from build123d import *

# Parameters (mm, degrees)
SKETCH_1_W      = 38
SKETCH_1_H      = 80
EXTRUDE_1_DEPTH = 4
SKETCH_2_W      = 38
SKETCH_2_H      = 8
EXTRUDE_2_DEPTH = 16


with BuildPart() as part:
    # 草图1 → 凸台-拉伸1 (new, symmetric)
    with BuildSketch(Plane.XY):
        Rectangle(SKETCH_1_W, SKETCH_1_H)
    extrude(amount=EXTRUDE_1_DEPTH, both=True)

    # 草图2 → 凸台-拉伸2 (add)
    with BuildSketch(Plane.XY.offset(4)):
        with Locations((0, 36)):
            Rectangle(SKETCH_2_W, SKETCH_2_H)
    extrude(amount=EXTRUDE_2_DEPTH)


solid = part.part
Work out the finished part from the listing and answer in its coordinate system (mm). A direction names the side the tool comes from. Coordinates: 2 decimals unless noted, no trailing zeros. Loops run counter-clockwise (first coordinate to the right, second up) from the corner with the lowest first, then second, coordinate; pieces in that order, holes last. Notation, with made-up numbers: M 46.5,35.25 L 90.5,35.25 A38 cw 90.5,74.25 Z; hole C -25,54 d9. An arc over 180 degrees is marked long. Answer in a Markdown table with one row per item. Add a question column.
1. A tool of negligible diameter and unlimited length cuts with its end or side. For faces 1 (the flat face through (0, 32, 12)), 2 (the flat face through (0, -40, 0)), from which of +Z, -Z, +X, -X, +Y, -Y can it reach the whole face along a straight path? Write none if from no direction.
2. Consider L1, parallel to Y at x = 3, z = 12.75; L2, parallel to Z at x = -4, y = -33. Determine where each line is inside the solid, lowest interval first.
3. Flat-ended cylindrical pins translate along their axes: P1, Ø8, axis at x = 11.5, y = -23, coming from the +Z side; P2, Ø1, axis at y = 12.5, z = 5, coming from the -X side; P3, Ø1, axis at x = -6.5, z = 8.5, coming from the -Y side. Find the tip coordinate at first contact, or state that the pin passes through.
4. Find section B-B, the plane y = -13. Write down the section's boundary in (x, z).
5. Find section A-A, the plane x = -11.5. Write down the section's boundary in (y, z), then the cut area to 3 significant figures.
6. Find section C-C, the plane z = 16.25. Write down the section's boundary in (x, y), then the cut area to 3 significant figures.
Reported:
| question | item | result |
|---|---|---|
| 1 | face 1 | +Z, +X, -X, -Y |
| 1 | face 2 | +Z, -Z, +X, -X, -Y |
| 2 | L1 | y = 32 to 40 |
| 2 | L2 | z = -4 to 4 |
| 3 | P1 | stops at z = 4 |
| 3 | P2 | passes through |
| 3 | P3 | stops at y = 32 |
| 4 | outline | M -19,-4 L 19,-4 L 19,4 L -19,4 Z |
| 5 | outline | M -40,-4 L 40,-4 L 40,20 L 32,20 L 32,4 L -40,4 Z |
| 5 | area | 768 mm^2 |
| 6 | outline | M -19,32 L 19,32 L 19,40 L -19,40 Z |
| 6 | area | 304 mm^2 |
